```python
from build123d import *

# Parameters (mm, degrees)
BASE_PLATE_SKETCH_W             = 150
BASE_PLATE_SKETCH_H             = 80
BASE_PLATE_SKETCH_R             = 12.5
BASE_PLATE_DEPTH                = 15
SKETCH1_4_R                     = 12.5
SKETCH1_4_R_2                   = 6
BASE_CONTOUR_EXTRUDE_10MM_DEPTH = 10
UPRIGHT_WALL_SKETCH_W           = 15
UPRIGHT_WALL_SKETCH_H           = 80
UPRIGHT_WALL_DEPTH              = 60
UPRIGHT_TOP_FILLET_R20_R        = 20
UPRIGHT_HOLES_SKETCH_R          = 7.5
UPRIGHT_MOUNTING_HOLES_DEPTH    = 40


with BuildPart() as part:
    # Base Plate Sketch → Base Plate (new body)
    with BuildSketch(Plane(origin=(0, 0, 0), x_dir=(1, 0, 0), z_dir=(0, 1, 0))):
        with Locations((75, 0)):
            Rectangle(BASE_PLATE_SKETCH_W, BASE_PLATE_SKETCH_H)
        with Locations(Location((74.768392371, 0, 0), (0, 0, 270))):
            Circle(BASE_PLATE_SKETCH_R, mode=Mode.SUBTRACT)
        with BuildLine():
            ThreePointArc((124.066474122, 28.46226077), (114.60740179, 30.996811562), (112.072850998, 21.53773923))
            ThreePointArc((112.072850998, 21.53773923), (117.843870831, 0), (112.072850998, -21.53773923))
            ThreePointArc((112.072850998, -21.53773923), (114.60740179, -30.996811562), (124.066474122, -28.46226077))
            ThreePointArc((124.066474122, -28.46226077), (131.69291391, 0), (124.066474122, 28.46226077))
        make_face(mode=Mode.SUBTRACT)
    extrude(amount=BASE_PLATE_DEPTH)

    # Sketch1_4 → Base Contour Extrude 10mm (add)
    with BuildSketch(Plane(origin=(0, 0, 0), x_dir=(1, 0, 0), z_dir=(0, 1, 0))):
        with Locations(Location((74.768392371, 0, 0), (0, 0, 270))):
            Circle(SKETCH1_4_R)
        with Locations(Location((74.768392371, 0, 0), (0, 0, 270))):
            Circle(SKETCH1_4_R_2, mode=Mode.SUBTRACT)
    extrude(amount=BASE_CONTOUR_EXTRUDE_10MM_DEPTH)

    # Upright Wall Sketch → Upright Wall (add)
    with BuildSketch(Plane(origin=(0, 15, 0), x_dir=(1, 0, 0), z_dir=(0, 1, 0))):
        with Locations((7.5, 0)):
            Rectangle(UPRIGHT_WALL_SKETCH_W, UPRIGHT_WALL_SKETCH_H)
    extrude(amount=UPRIGHT_WALL_DEPTH)

    # Upright Top Fillet R20
    upright_top_fillet_r20_edges = [part.edges().sort_by_distance(p)[0] for p in [
        (7.5, 75, 40),
        (7.5, 75, -40),
    ]]
    fillet(upright_top_fillet_r20_edges, radius=UPRIGHT_TOP_FILLET_R20_R)

    # Upright Holes Sketch → Upright Mounting Holes (cut, symmetric)
    with BuildSketch(Plane(origin=(15, 0, 0), x_dir=(0, 0, -1), z_dir=(1, 0, 0))):
        with Locations((20, 55)):
            Circle(UPRIGHT_HOLES_SKETCH_R)
        with Locations((-20, 55)):
            Circle(UPRIGHT_HOLES_SKETCH_R)
    extrude(amount=UPRIGHT_MOUNTING_HOLES_DEPTH, both=True, mode=Mode.SUBTRACT)


solid = part.part
```
Geometry check sheet. Reference: the model listing, model coordinates, mm. A direction names the side the tool comes from. Coordinates: 2 decimals unless noted, no trailing zeros. Write each loop counter-clockwise with the first axis right and the second up, starting at its lowest first coordinate (ties: lowest second). Pieces come first, ordered by that corner, then holes. Notation, with made-up numbers: M 86,83 L 100,83 A21 cw 100,115 Z; hole C 68,-6 d2. An arc over 180 degrees is marked long. Use one line per item in the form item = value. Start each with the question number.
1) Release check for a two-part mould opening along Z. For faces 4 (the flat face through (57, 9, -40)), 5 (the flat face through (57, 9, 40)), 6 (the flat face through (150, 7, 1)), 7 (the cylindrical face through (114.48, 7.4, 30.92)) record: pulls with the +Z half, pulls with the -Z half, needs draft (parallel to the pull), parting line crosses it, or undercut.
2) Go/stop test with flat-tipped pins: pin 1 Ø19.5 at (y, z) = (55, -20) entering from +X; pin 2 Ø12.5 at (x, z) = (78.5, -1.5) entering from +Y; pin 3 Ø4 at (x, z) = (119.5, -28) entering from +Y; pin 4 Ø24 at (x, z) = (56, 8) entering from +Y. Record where each tip stops, or that it passes through.
3) Section check D-D on y = 7. Enter the section's corners in (x, z).
4) Section check B-B on y = 59.5. Enter the section's corners in (x, z).
5) Thickness scan on probe 1 along X at (y, z) = (2, 0); probe 2 along X at (y, z) = (14, 7.5); probe 3 along Y at (x, z) = (10, -20). Record the ranges inside material, lowest first. Write a range as from..to.
6) Section check A-A on z = 0. Enter the section's corners in (x, y).
7) Section check C-C on z = 8. Enter the section's corners in (x, y), and give its area (3 significant figures).
8) Set-up check for faces 1 (the cylindrical face through (131.69, 7.4, 0.42)), 2 (the flat face through (69, 10, -3)), 3 (the flat face through (15, 45, 1)): record each of +Z, -Z, +X, -X, +Y, -Y from which the full face is reachable in a straight line by a thin tool's end or side.
Responses:
q1.face_4 = pulls with the -Z half
q1.face_5 = pulls with the +Z half
q1.face_6 = needs draft
q1.face_7 = undercut
q2.pin_1 = 15
q2.pin_2 = 10
q2.pin_3 = through
q2.pin_4 = 15
q3.outline = M 0,-40 L 150,-40 L 150,40 L 0,40 Z; hole C 74.77,0 d12; hole M 112.07,-21.54 A6.92 ccw 124.07,-28.46 A56.92 ccw 124.07,28.46 A6.92 ccw 112.07,21.54 A43.08 cw Z
q4.outline = M 0,-39.49 L 15,-39.49 L 15,-26 L 0,-26 Z; M 0,-14 L 15,-14 L 15,14 L 0,14 Z; M 0,26 L 15,26 L 15,39.49 L 0,39.49 Z
q5.probe_1 = 0..68.77, 80.77..117.84, 131.69..150
q5.probe_2 = 0..64.77, 84.77..117.19, 131.2..150
q5.probe_3 = 0..47.5, 62.5..75
q6.outline = M 0,0 L 68.77,0 L 68.77,10 L 62.27,10 L 62.27,15 L 15,15 L 15,75 L 0,75 Z; M 80.77,0 L 117.84,0 L 117.84,15 L 87.27,15 L 87.27,10 L 80.77,10 Z; M 131.69,0 L 150,0 L 150,15 L 131.69,15 Z
q7.outline = M 0,0 L 117.09,0 L 117.09,15 L 84.37,15 L 84.37,10 L 65.16,10 L 65.16,15 L 15,15 L 15,75 L 0,75 Z; M 131.13,0 L 150,0 L 150,15 L 131.13,15 Z
q7.area = 2,840 mm2
q8.face_1 = +Y, -Y
q8.face_2 = +Y
q8.face_3 = +Z, -Z, +X, +Y
